from build123d import *

# Parameters (mm, degrees)
SKETCH1_W          = 2
SKETCH1_H          = 20
SKETCH2_R          = 4
CUT_EXTRUDE1_DEPTH = 10
SCALE_1_SCALE      = 1.875


with BuildPart() as part:
    # Sketch1 → Revolve1 (revolve)
    with BuildSketch(Plane.XY, mode=Mode.PRIVATE) as revolve1_sk:
        with Locations((1, 46)):
            Rectangle(SKETCH1_W, SKETCH1_H)
    revolve(revolve1_sk.sketch.rotate(Axis((0, 0, 0), (1, 0, 0)), 90), axis=Axis((0, 0, 0), (1, 0, 0)))

    # Sketch2 → Cut-Extrude1 (cut)
    with BuildSketch(Plane(origin=(2, 0, 0), x_dir=(0, 0, -1), z_dir=(1, 0, 0))):
        with Locations((0, 46)):
            Circle(SKETCH2_R)
        with Locations((39.837168574, 23)):
            Circle(SKETCH2_R)
        with Locations((-39.837168574, 23)):
            Circle(SKETCH2_R)
        with Locations((-39.837168574, -23)):
            Circle(SKETCH2_R)
        with Locations((0, -46)):
            Circle(SKETCH2_R)
        with Locations((39.837168574, -23)):
            Circle(SKETCH2_R)
    extrude(amount=-CUT_EXTRUDE1_DEPTH, mode=Mode.SUBTRACT)


with BuildPart() as part_1:
    # Scale 1: scaled about (1, 0, 0)
    add(part.part.scale(SCALE_1_SCALE).moved(Location((-0.875, 0, 0))))


solid = part_1.part
Read the model definition and answer for the solid it produces. Units are mm, in the model's axes. Coordinates: 2 decimals unless noted, no trailing zeros. Write each loop counter-clockwise with the first axis right and the second up, starting at its lowest first coordinate (ties: lowest second). Pieces come first, ordered by that corner, then holes. Notation, with made-up numbers: M -0.75,26.25 L 6.25,26.25 A30 ccw 6.25,57.25 Z; hole C 42,83 d8. An arc over 180 degrees is marked long. Use a Markdown table: item, result.
Q1. The part is cut by section D-D, the plane x = 0.15. Write down the section's boundary in (y, z) (3 decimals), then the cut area to 3 significant figures.
Answer block:
| item | result |
|---|---|
| outline | C 0,0 d210; hole C -86.25,0 d15; hole C 0,0 d135; hole C -43.125,-74.695 d15; hole C -43.125,74.695 d15; hole C 43.125,-74.695 d15; hole C 43.125,74.695 d15; hole C 86.25,0 d15 |
| area | 19,300 mm2 |
Q2. Determine the mould class of faces 1 (the face through (2.875, -1, -69)), 2 (the face through (1.026, -50.447, 76.321)), 3 (the face through (1.03, -31.54, 100.15)) for opening direction Y: released by +Y, released by -Y, zero draft, split by the parting line, or undercut.
Answer block:
| item | result |
|---|---|
| face 1 | zero draft |
| face 2 | undercut |
| face 3 | split by the parting line |
Q3. Straight lines are drawn through the part: L1, parallel to Y at x = 0.5, z = 0; L2, parallel to Z at x = 0.6, y = 50; L3, parallel to Z at x = -0.5, y = 46. For each, find the intervals that lie inside material, in ascending order. Write a range as [from, to].
Answer block:
| item | result |
|---|---|
| L1 | y = [-105, -93.75], [-78.75, -67.5], [67.5, 78.75], [93.75, 105] |
| L2 | z = [-92.33, -77.69], [-71.7, -45.35], [45.35, 71.7], [77.69, 92.33] |
| L3 | z = [-94.39, -81.62], [-67.77, -49.4], [49.4, 67.77], [81.62, 94.39] |
Q4. The part is cut by section A-A, the plane z = 0. Write down the section's boundary in (x, y) (3 decimals).
Answer block:
| item | result |
|---|---|
| outline | M -0.875,-105 L 2.875,-105 L 2.875,-93.75 L -0.875,-93.75 Z; M -0.875,-78.75 L 2.875,-78.75 L 2.875,-67.5 L -0.875,-67.5 Z; M -0.875,67.5 L 2.875,67.5 L 2.875,78.75 L -0.875,78.75 Z; M -0.875,93.75 L 2.875,93.75 L 2.875,105 L -0.875,105 Z |
Q5. The part is cut by section C-C, the plane z = -33. Write down the section's boundary in (x, y) (3 decimals), then the cut area to 3 significant figures.
Answer block:
| item | result |
|---|---|
| outline | M -0.875,-99.679 L 2.875,-99.679 L 2.875,-58.883 L -0.875,-58.883 Z; M -0.875,58.883 L 2.875,58.883 L 2.875,99.679 L -0.875,99.679 Z |
| area | 306 mm2 |
Q6. The part is cut by section B-B, the plane y = 0. Write down the section's boundary in (x, z) (3 decimals), then the cut area to 3 significant figures.
Answer block:
| item | result |
|---|---|
| outline | M -0.875,-105 L 2.875,-105 L 2.875,-67.5 L -0.875,-67.5 Z; M -0.875,67.5 L 2.875,67.5 L 2.875,105 L -0.875,105 Z |
| area | 281 mm2 |
